Design review of the part built by this model. Coordinates are the model's own, in mm. A direction names the side the tool comes from. Round coordinates to 2 decimals unless told otherwise and drop trailing zeros. Loops run counter-clockwise (first coordinate to the right, second up) from the corner with the lowest first, then second, coordinate; pieces in that order, holes last. Notation, with made-up numbers: M 53,22 L 78,22 A12 cw 78,37 Z; hole C 67,-25 d2. An arc over 180 degrees is marked long. Answer as CSV lines item,"result". Start each with the question number.
from build123d import *

# Parameters (mm, degrees)
SKETCH1_W                                           = 80
SKETCH1_H                                           = 25
BOSS_EXTRUDE1_DEPTH                                 = 12
SKETCH2_W                                           = 10
SKETCH2_H                                           = 2
CUT_EXTRUDE1_DEPTH                                  = 49.672374095
CBORE_FOR_M5_HEX_SOCKET_HEAD_CAP_SCREW1_D           = 5.5
CBORE_FOR_M5_HEX_SOCKET_HEAD_CAP_SCREW1_CBORE_D     = 10
CBORE_FOR_M5_HEX_SOCKET_HEAD_CAP_SCREW1_CBORE_DEPTH = 5.4
CBORE_FOR_M5_HEX_SOCKET_HEAD_CAP_SCREW2_D           = 5.5
CBORE_FOR_M5_HEX_SOCKET_HEAD_CAP_SCREW2_CBORE_D     = 10
CBORE_FOR_M5_HEX_SOCKET_HEAD_CAP_SCREW2_CBORE_DEPTH = 5.4


with BuildPart() as part:
    # Sketch1 → Boss-Extrude1 (new body)
    with BuildSketch(Plane.XY):
        Rectangle(SKETCH1_W, SKETCH1_H)
    extrude(amount=BOSS_EXTRUDE1_DEPTH)

    # Sketch2 → Cut-Extrude1 (cut, through all)
    with BuildSketch(Plane(origin=(0, 12.5, 0), x_dir=(1, 0, 0), z_dir=(0, 1, 0))):
        with Locations((-30, -1)):
            Rectangle(SKETCH2_W, SKETCH2_H)
        with Locations((-3, -1)):
            Rectangle(SKETCH2_W, SKETCH2_H)
        with Locations((30, -1)):
            Rectangle(SKETCH2_W, SKETCH2_H)
    extrude(amount=-CUT_EXTRUDE1_DEPTH, mode=Mode.SUBTRACT)

    # CBORE for M5 Hex Socket Head Cap Screw1 (through all)
    with Locations(Plane.XY.offset(12)):
        with Locations((-30, 7), (-30, -7), (-3, 7), (-3, -7), (30, 7), (30, -7)):
            CounterBoreHole(CBORE_FOR_M5_HEX_SOCKET_HEAD_CAP_SCREW1_D / 2, CBORE_FOR_M5_HEX_SOCKET_HEAD_CAP_SCREW1_CBORE_D / 2, CBORE_FOR_M5_HEX_SOCKET_HEAD_CAP_SCREW1_CBORE_DEPTH)

    # CBORE for M5 Hex Socket Head Cap Screw2 (through all)
    with Locations(Plane(origin=(0, 0, 0), x_dir=(-1, 0, 0), z_dir=(0, 0, -1))):
        with Locations((-13.5, 6.5), (-13.5, -6.5), (16.5, 6.5), (16.5, -6.5)):
            CounterBoreHole(CBORE_FOR_M5_HEX_SOCKET_HEAD_CAP_SCREW2_D / 2, CBORE_FOR_M5_HEX_SOCKET_HEAD_CAP_SCREW2_CBORE_D / 2, CBORE_FOR_M5_HEX_SOCKET_HEAD_CAP_SCREW2_CBORE_DEPTH)


solid = part.part
Item 1: Consider section B-B, the plane x = -16.5. Write out the cut boundary in (y, z).
Item 2: Consider section D-D, the plane x = 29.5. Write out the cut boundary in (y, z).
Item 3: Insertion check: pin 1 Ø3 at (x, y) = (-5.5, -5) entering from +Z; pin 2 Ø5 at (x, y) = (14, -7.5) entering from -Z; pin 3 Ø4.5 at (x, y) = (-30, 7) entering from -Z; pin 4 Ø9 at (x, y) = (30, 7) entering from -Z. Each pin has a flat end and moves straight along its axis. Give the tip position at first contact, or say it passes through.
Item 4: Consider section A-A, the plane z = 9.5. Count the separate pieces of the cut face and the enclosed holes in it, then the cut area to 3 significant figures.
Item 5: Tool access review of faces 4 (the face through (-19, -9, 5.4)), 5 (the face through (-27.8, 4.8, 6.6)), 6 (the face through (-18.682, 4.827, 8.746)), 7 (the face through (2, 0, 1)): name each direction out of +Z, -Z, +X, -X, +Y, -Y from which nothing blocks a thin tool from reaching the whole face with its end or side.
Item 6: To check wall thickness, follow line 1 (Y direction, x = -16.5, z = 3.85); line 2 (Y direction, x = 30, z = 3); line 3 (X direction, y = 2.25, z = 4.5). State the ranges of each line that lie inside material, in increasing order.
Item 7: The part is to be moulded in two halves that separate along Y. For faces 1 (the face through (25, -7, 9)), 2 (the face through (-25, 0, 1)), 3 (the face through (-1, -12.5, 6)), say which applies: +Y half, -Y half, draft (parallel to the pull), parting line (faces both ways), or undercut.
Found:
1,outline,"M -12.5,0 L -11.5,0 L -11.5,5.4 L -9.25,5.4 L -9.25,12 L -12.5,12 Z; M -3.75,5.4 L -1.5,5.4 L -1.5,0 L 1.5,0 L 1.5,5.4 L 3.75,5.4 L 3.75,12 L -3.75,12 Z; M 9.25,5.4 L 11.5,5.4 L 11.5,0 L 12.5,0 L 12.5,12 L 9.25,12 Z"
2,outline,"M -12.5,2 L -9.7,2 L -9.7,6.6 L -11.97,6.6 L -11.97,12 L -12.5,12 Z; M -4.3,2 L 4.3,2 L 4.3,6.6 L 2.03,6.6 L 2.03,12 L -2.03,12 L -2.03,6.6 L -4.3,6.6 Z; M 9.7,2 L 12.5,2 L 12.5,12 L 11.97,12 L 11.97,6.6 L 9.7,6.6 Z"
3,pin 1,"stops at z = 6.6"
3,pin 2,"stops at z = 5.4"
3,pin 3,"passes through"
3,pin 4,"stops at z = 2"
4,separate pieces,"1"
4,enclosed holes,"10"
4,area,"1,430 mm^2"
5,face 4,"-Z"
5,face 5,"+Z"
5,face 6,"+Z, -Z"
5,face 7,"-Z, +Y, -Y"
6,line 1,"y = -12.5 to -11.5, -1.5 to 1.5, 11.5 to 12.5"
6,line 2,"y = -12.5 to -9.75, -4.25 to 4.25, 9.75 to 12.5"
6,line 3,"x = -40 to -19.13, -13.87 to 10.87, 16.13 to 40"
7,face 1,"undercut"
7,face 2,"draft"
7,face 3,"-Y half"
